Part model, mm, in its own coordinate system. A direction names the side the tool comes from. Give positions to 0.01 mm unless a question says otherwise; leave off trailing zeros. Write each loop counter-clockwise with the first axis right and the second up, starting at its lowest first coordinate (ties: lowest second). Pieces come first, ordered by that corner, then holes. Notation, with made-up numbers: (19.5, 31.25) - (56.5, 31.25) arc R10 cw to (56.5, 38.25) - close; hole circle Ø6 at (-4.75, 44.25). An arc over 180 degrees is marked (long way). Answer as a JSON object with one key per item and string values. Group by question number.
```python
from build123d import *


with BuildPart() as part:
    # Sketch1 → Revolve1 (revolve)
    with BuildSketch(Plane.XY, mode=Mode.PRIVATE) as revolve1_sk:
        Polygon((0, 40), (-12, 40), (-12, 14), (-12.5, 14), (-12.5, 8), (-10, 8), (-10, 0), (0, 0), align=None)
    revolve(revolve1_sk.sketch.rotate(Axis((0, 0, 0), (0, 1, 0)), 270), axis=Axis((0, 0, 0), (0, 1, 0)))


solid = part.part
```
1) Saw through at C-C (y = 19). List the corners of the cut face in (x, z), and give its area (3 significant figures).
2) Saw through at A-A (z = 0). List the corners of the cut face in (x, y).
3) Which spindle directions (+Z, -Z, +X, -X, +Y, -Y) get a long thin tool onto all of the face, cutting with end or side? Do faces 1 (the cylindrical face through (9.76, 3.94, 2.17)), 2 (the cylindrical face through (-3.755, 10.958, -11.923)), 3 (the cylindrical face through (-3.604, 26.818, -11.446)). Say none if no direction does.
4) Saw through at D-D (x = 10.75). List the corners of the cut face in (y, z), and give its area (3 significant figures).
5) Saw through at B-B (x = 0). List the corners of the cut face in (y, z).
6) Drill centre lines: line 1 along Y through (x, z) = (-5.75, -8.5); line 2 along Z through (x, y) = (3.75, 19.5); line 3 along X through (y, z) = (2, 4). Where is each one in solid material? Low to high. Write a range as from..to.
7) Drop flat-ended pins along their axis: P1, Ø1.5, axis at x = -1, z = -0.5, coming from the -Y side; P2, Ø2, axis at y = 13.5, z = -7.5, coming from the +X side; P3, Ø2, axis at x = 8, y = 33, coming from the -Z side; P4, Ø12, axis at x = -1, y = 29.5, coming from the -Z side. Give the stop position or say it passes through.
Checks:
{
 "1": {"outline": "circle Ø24 at (0, 0)", "area": "452 mm2"},
 "2": {"outline": "(-12.5, 8) - (-10, 8) - (-10, 0) - (10, 0) - (10, 8) - (12.5, 8) - (12.5, 14) - (12, 14) - (12, 40) - (-12, 40) - (-12, 14) - (-12.5, 14) - close"},
 "3": {"face 1": "-Y", "face 2": "+Y, -Y", "face 3": "+Y"},
 "4": {"outline": "(8, -6.38) - (14, -6.38) - (14, -5.33) - (40, -5.33) - (40, 5.33) - (14, 5.33) - (14, 6.38) - (8, 6.38) - close", "area": "354 mm2"},
 "5": {"outline": "(0, -10) - (8, -10) - (8, -12.5) - (14, -12.5) - (14, -12) - (40, -12) - (40, 12) - (14, 12) - (14, 12.5) - (8, 12.5) - (8, 10) - (0, 10) - close"},
 "6": {"line 1": "8..40", "line 2": "-11.4..11.4", "line 3": "-9.17..9.17"},
 "7": {"P1": "y = 0", "P2": "x = 10.68", "P3": "z = -9.75", "P4": "z = -12"}
}
